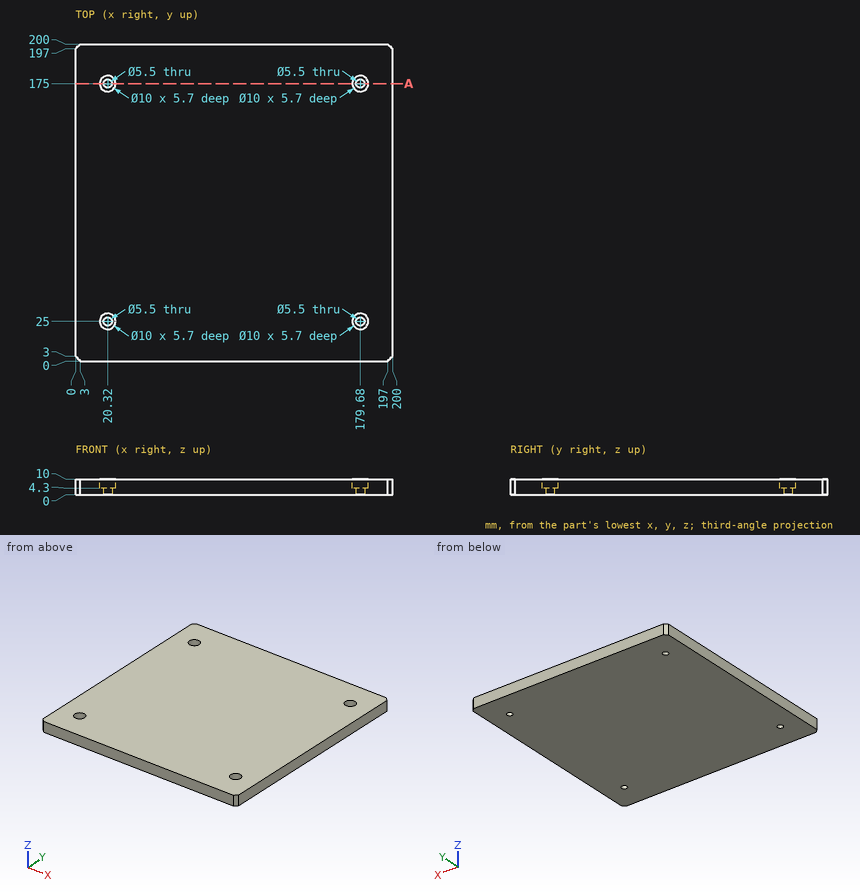
The figure shows three views and two pictorial views of one solid part (mm, origin at its lowest corner). Answer the questions. Round coordinates to 2 decimals unless told otherwise and drop trailing zeros. Loops run counter-clockwise (first coordinate to the right, second up) from the corner with the lowest first, then second, coordinate; pieces in that order, holes last. Notation, with made-up numbers: (-35, -6) - (-18, -6) arc R29 cw to (-18, 28) - close; hole circle Ø6 at (87.5, 60). An arc over 180 degrees is marked (long way). One line per question, with ' | ' between items. Start each with the question number.
Q1. Section A-A on y = 175 is taken. Give the vertices of the cut face in (x, z).
Q2. Flat-ended cylindrical pins translate along their axes: pin 1 (6.5 mm diameter, centred on x = 179.68, y = 25, fed in from +Z); pin 2 (3.5 mm diameter, centred on x = 179.68, y = 175, fed in from -Z). Find the tip coordinate at first contact, or state that the pin passes through.
Q3. Find the intervals of material crossed by L1, parallel to X at y = 175, z = 7.05; L2, parallel to X at y = 175, z = 1.4, in increasing order.
Established:
1) outline: (0, 0) - (17.57, 0) - (17.57, 4.3) - (15.32, 4.3) - (15.32, 10) - (0, 10) - close; (23.07, 0) - (176.93, 0) - (176.93, 4.3) - (174.68, 4.3) - (174.68, 10) - (25.32, 10) - (25.32, 4.3) - (23.07, 4.3) - close; (182.43, 0) - (200, 0) - (200, 10) - (184.68, 10) - (184.68, 4.3) - (182.43, 4.3) - close
2) pin 1: z = 4.3 | pin 2: through
3) L1: 0 to 15.32, 25.32 to 174.68, 184.68 to 200 | L2: 0 to 17.57, 23.07 to 176.93, 182.43 to 200
